Geometry: final body of the model. Coordinates: model frame, mm. Face numbers are marked on the shaded views. A direction names the side the tool comes from. Coordinates: 2 decimals unless noted, no trailing zeros. Write each loop counter-clockwise with the first axis right and the second up, starting at its lowest first coordinate (ties: lowest second). Pieces come first, ordered by that corner, then holes. Notation, with made-up numbers: M -10,71.25 L 20,71.25 A31 ccw 20,106.25 Z; hole C 59.5,-39 d7. An arc over 180 degrees is marked long. Write item = value, one per line. Start each with the question number.
Item 1: Section B-B on x = 6. Output: boundary loops of the cut face in (y, z).
Item 2: Pull-direction query (Y, two-part tool) for the marked faces 1, 2 and 3; classes: +Y half, -Y half, draft (parallel to the pull), parting line (faces both ways), or undercut.
Item 3: Section A-A on z = 0. Output: boundary loops of the cut face in (x, y), plus the area to 3 significant figures.
Item 4: Section D-D on y = 0. Output: boundary loops of the cut face in (x, z), plus the area to 3 significant figures.
Item 5: First-contact query: pin 1 Ø1 at (y, z) = (-5, -6.5) entering from +X; pin 2 Ø3 at (x, y) = (-7.5, -9.5) entering from -Z; pin 3 Ø6.5 at (y, z) = (-19, -0.5) entering from -X. Flat tips, straight axial feed; report the tip coordinate or a pass-through.
Item 6: Reachability of the marked faces 4, 5, 6, 7 and 8 from +Z, -Z, +X, -X, +Y, -Y: full face, straight path, thin tool, end or side. Return the list, or none.
Item 7: Ray query, L1, parallel to X at y = -17.5, z = 0; L2, parallel to Z at x = -29, y = 4; L3, parallel to Y at x = -63, z = -18. Return the intervals inside material, ascending. Write a range as [from, to].
Item 8: Section C-C on x = -4.5. Output: boundary loops of the cut face in (y, z).
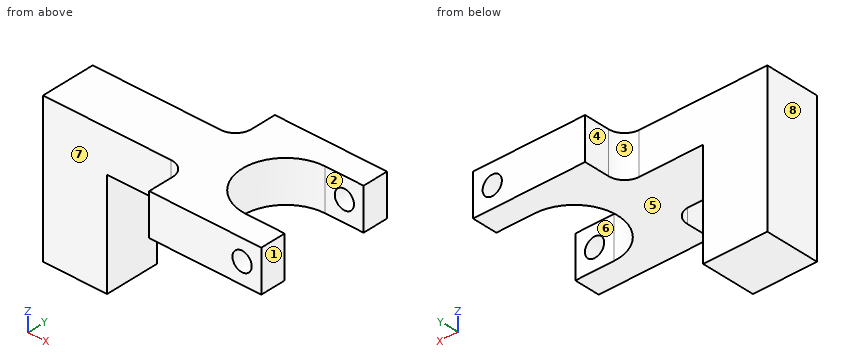
from build123d import *

# Parameters (mm, degrees)
EXTRUDE_1_DEPTH     = 6.5
CUT_EXTRUDE_1_REACH = 74.493
SKETCH_2_W          = 45
SKETCH_2_H          = 13
FILLET_1_R          = 5
SKETCH_3_W          = 20
SKETCH_3_H          = 17
EXTRUDE_2_DEPTH     = 33
CUT_EXTRUDE_2_REACH = 91.628
SKETCH_4_R          = 3


with BuildPart() as part:
    # 草图1 → 凸台-拉伸1 (new, symmetric)
    with BuildSketch(Plane.XY):
        with BuildLine():
            Line((0, 13.5), (12, 13.5))
            Line((12, 13.5), (12, 21.5))
            Line((12, 21.5), (-68, 21.5))
            Line((-68, 21.5), (-68, -21.5))
            Line((-68, -21.5), (12, -21.5))
            Line((12, -21.5), (12, -13.5))
            Line((12, -13.5), (0, -13.5))
            ThreePointArc((0, -13.5), (-13.5, 0), (0, 13.5))
        make_face()
    extrude(amount=EXTRUDE_1_DEPTH, both=True)

    # 草图2 → 切除-拉伸1 (cut, up to next)
    with BuildSketch(Plane.XY.offset(6.5), mode=Mode.PRIVATE) as cut_extrude_1_sk1:
        with Locations((-45.5, 15)):
            Rectangle(SKETCH_2_W, SKETCH_2_H)
    cut_extrude_1_tool1 = extrude(cut_extrude_1_sk1.sketch, amount=-CUT_EXTRUDE_1_REACH, mode=Mode.PRIVATE) & part.part
    # 草图2 → 切除-拉伸1 (cut, up to next)
    with BuildSketch(Plane.XY.offset(6.5), mode=Mode.PRIVATE) as cut_extrude_1_sk2:
        with Locations((-45.5, -15)):
            Rectangle(SKETCH_2_W, SKETCH_2_H)
    cut_extrude_1_tool2 = extrude(cut_extrude_1_sk2.sketch, amount=-CUT_EXTRUDE_1_REACH, mode=Mode.PRIVATE) & part.part
    add(cut_extrude_1_tool1.solids().sort_by_distance((-45.5, 15, 6.5))[0], mode=Mode.SUBTRACT)
    add(cut_extrude_1_tool2.solids().sort_by_distance((-45.5, -15, 6.5))[0], mode=Mode.SUBTRACT)

    # 圆角1
    fillet_1_edges = [part.edges().sort_by_distance(p)[0] for p in [
        (-23, 8.5, 0),
        (-23, -8.5, 0),
    ]]
    fillet(fillet_1_edges, radius=FILLET_1_R)

    # 草图3 → 凸台-拉伸2 (add)
    with BuildSketch(Plane(origin=(0, 0, -6.5), x_dir=(-1, 0, 0), z_dir=(0, 0, -1))):
        with Locations((58, 0)):
            Rectangle(SKETCH_3_W, SKETCH_3_H)
    extrude(amount=EXTRUDE_2_DEPTH)

    # 切除-拉伸2: up to this face of the body (flat: up to its plane)
    cut_extrude_2_end = Plane(part.part.faces().sort_by_distance((-5.5, 21.5, 0))[0])
    # 草图4 → 切除-拉伸2 (cut, up to the picked face)
    with BuildSketch(Plane.XZ.offset(21.5), mode=Mode.PRIVATE) as cut_extrude_2_sk1:
        with Locations(Location((6, 0, 0), (0, 0, 270))):
            Circle(SKETCH_4_R)
    cut_extrude_2_tool1 = split(extrude(cut_extrude_2_sk1.sketch, amount=-CUT_EXTRUDE_2_REACH, mode=Mode.PRIVATE), bisect_by=cut_extrude_2_end, keep=Keep.BOTH, mode=Mode.PRIVATE)
    add(cut_extrude_2_tool1.solids().sort_by(Axis((6, -21.5, 0), (0, 1, 0)))[0], mode=Mode.SUBTRACT)


solid = part.part
Responses:
q1.outline = M -21.5,-6.5 L -13.5,-6.5 L -13.5,-3 L -21.5,-3 Z; M -21.5,3 L -13.5,3 L -13.5,6.5 L -21.5,6.5 Z; M 13.5,-6.5 L 21.5,-6.5 L 21.5,-3 L 13.5,-3 Z; M 13.5,3 L 21.5,3 L 21.5,6.5 L 13.5,6.5 Z
q2.face_1 = draft
q2.face_2 = undercut
q2.face_3 = +Y half
q3.outline = M -68,-8.5 L -28,-8.5 A5 cw -23,-13.5 L -23,-21.5 L 3,-21.5 L 3,-13.5 L 0,-13.5 A13.5 cw 0,13.5 L 3,13.5 L 3,21.5 L -23,21.5 L -23,13.5 A5 cw -28,8.5 L -68,8.5 Z; M 9,-21.5 L 12,-21.5 L 12,-13.5 L 9,-13.5 Z; M 9,13.5 L 12,13.5 L 12,21.5 L 9,21.5 Z
q3.area = 1,570 mm²
q4.outline = M -68,-39.5 L -48,-39.5 L -48,-6.5 L -13.5,-6.5 L -13.5,6.5 L -68,6.5 Z
q4.area = 1,370 mm²
q5.pin_1 = -12.33
q5.pin_2 = -6.5
q5.pin_3 = -23
q6.face_4 = +Z, -Z, -X, +Y
q6.face_5 = -Z, +X, +Y, -Y
q6.face_6 = +Z, -Z, +X
q6.face_7 = +Z, -Z, -X, -Y
q6.face_8 = +Z, -Z, -X, +Y, -Y
q7.L1 = [-23, 3], [9, 12]
q7.L2 = [-6.5, 6.5]
q7.L3 = [-8.5, 8.5]
q8.outline = M -21.5,-6.5 L -12.73,-6.5 L -12.73,6.5 L -21.5,6.5 Z; M 12.73,-6.5 L 21.5,-6.5 L 21.5,6.5 L 12.73,6.5 Z
